Geometry check sheet. Reference: the model listing, model coordinates, mm. A direction names the side the tool comes from. Give positions to 0.01 mm unless a question says otherwise; leave off trailing zeros. Loops run counter-clockwise (first coordinate to the right, second up) from the corner with the lowest first, then second, coordinate; pieces in that order, holes last.
1. Material ranges on L1, parallel to Y at x = 805, z = 15; L2, parallel to Y at x = 805, z = 49.1; L3, parallel to X at y = 87, z = 7, recorded low to high.
2. Cross-section at A-A, the plane z = 12. State how many separate pieces and enclosed holes the cut face has, plus the area to 3 significant figures.
3. Cross-section at D-D, the plane x = 525.5. Record the cut outline in (y, z).
4. Go/stop test with a flat-tipped pin: pin 1 Ø10 at (y, z) = (197, 32) entering from -X. Record where the tip stops, or that it passes through.
5. Cross-section at B-B, the plane x = -600. Record the cut outline in (y, z), plus the area to 3 significant figures.
6. Release check for a two-part mould opening along Y. For faces 1 (the flat face through (113, 1010, 25)), 2 (the flat face through (92, 624, 0)), 3 (the cylindrical face through (-330.382, 940.039, 23.664)), 4 (the flat face through (-5, 0, 25)) record: +Y half, -Y half, draft (parallel to the pull), parting line (faces both ways), or undercut.
7. Tool access check on faces 5 (the flat face through (-512, 410, 25)), 6 (the flat face through (609, 410, 25)), 7 (the cylindrical face through (-563.05, 944.68, 49.01)), 8 (the cylindrical face through (809.878, 938.035, 23.664)). Record the directions out of +Z, -Z, +X, -X, +Y, -Y that give a thin tool (end or side, any length) a straight path to the whole face; none if there is none.
from build123d import *

# Parameters (mm, degrees)
BOSS_EXTRUDE1_DEPTH = 50
HOLE1_D             = 45
HOLE1_CBORE_D       = 80
HOLE1_CBORE_DEPTH   = 2
CHAMFER1_SIZE       = 20


with BuildPart() as part:
    # Sketch1 → Boss-Extrude1 (new body)
    with BuildSketch(Plane.XY):
        Polygon((390, 410), (855, 410), (855, 1010), (-650, 1010), (-650, 410), (-390, 410), (-390, 0), (390, 0), align=None)
    extrude(amount=BOSS_EXTRUDE1_DEPTH)

    # Hole1 (through all)
    with Locations(Plane.XY.offset(50)):
        with Locations((-600, 960), (320, 960), (805, 960), (-340, 60), (340, 60), (-320, 960), (805, 460), (320, 460), (-320, 460), (-600, 460)):
            CounterBoreHole(HOLE1_D / 2, HOLE1_CBORE_D / 2, HOLE1_CBORE_DEPTH)

    # Chamfer1
    chamfer1_edges = [part.edges().sort_by_distance(p)[0] for p in [
        (-650, 410, 25),
        (-650, 1010, 25),
        (855, 1010, 25),
        (855, 410, 25),
        (390, 0, 25),
        (-390, 0, 25),
    ]]
    chamfer(chamfer1_edges, length=CHAMFER1_SIZE)


solid = part.part
Result:
1. L1: y = 410 to 437.5, 482.5 to 937.5, 982.5 to 1010
1. L2: y = 410 to 420, 500 to 920, 1000 to 1010
1. L3: x = -390 to 390
2. separate pieces: 1
2. enclosed holes: 10
2. area: 1,210,000 mm2
3. outline: (410, 0) - (1010, 0) - (1010, 50) - (410, 50) - close
4. pin 1: stops at x = -390
5. outline: (410, 0) - (437.5, 0) - (437.5, 48) - (420, 48) - (420, 50) - (410, 50) - close; (482.5, 0) - (937.5, 0) - (937.5, 48) - (920, 48) - (920, 50) - (500, 50) - (500, 48) - (482.5, 48) - close; (982.5, 0) - (1010, 0) - (1010, 50) - (1000, 50) - (1000, 48) - (982.5, 48) - close
5. area: 25,400 mm2
6. face 1: +Y half
6. face 2: draft
6. face 3: undercut
6. face 4: -Y half
7. face 5: +Z, -Z, -X, -Y
7. face 6: +Z, -Z, +X, -Y
7. face 7: +Z
7. face 8: +Z, -Z
